Part model, mm, in its own coordinate system. A direction names the side the tool comes from. Round coordinates to 2 decimals unless told otherwise and drop trailing zeros. Order: outer loops, then holes, each group sorted by start corner. A loop starts at its lowest first (then second) coordinate and runs counter-clockwise, first axis right, second up. Notation, with made-up numbers: (74.25, -17) -> (117.25, -17) arc R12 cw to (117.25, -10) -> close; hole circle Ø10 at (38.25, 72). An arc over 180 degrees is marked (long way). Answer as a JSON object with one key per item and string values. Group by question number.
```python
from build123d import *

# Parameters (mm, degrees)
BRACKET_PLATE_DEPTH        = 10
UPPER_PIVOT_BOSS_DEPTH     = 13.5
UPPER_PIVOT_BORE_PROFILE_R = 9
UPPER_PIVOT_BORE_18_DEPTH  = 27
LOWER_PIVOT_BOSS_DEPTH     = 13.5
LOWER_PIVOT_BORE_PROFILE_R = 10
LOWER_PIVOT_BORE_20_DEPTH  = 27
STOP_LUG_DEPTH             = 13.5
PLATE_FILLET_R10_R         = 10


with BuildPart() as part:
    # Bracket Plate Profile → Bracket Plate (new body)
    with BuildSketch(Plane.XY):
        with BuildLine():
            Line((-32, 0), (-32, -68))
            Line((-32, -68), (0, -106.5))
            Line((0, -106.5), (116.5, -106.5))
            Line((116.5, -106.5), (116.5, -58.5))
            Line((116.5, -58.5), (88.5, -58.5))
            Line((88.5, -58.5), (88.5, -68.5))
            ThreePointArc((88.5, -68.5), (83.524922359, -76.549844719), (74.1, -75.7))
            Line((74.1, -75.7), (23.7, -37.9))
            ThreePointArc((23.7, -37.9), (21.602252409, -35.552292952), (20.572822936, -32.576969725))
            Line((20.572822936, -32.576969725), (15.854354129, 2.15393945))
            ThreePointArc((15.854354129, 2.15393945), (10.524660774, 12.051203907), (0, 16))
            Line((0, 16), (0, 32))
            ThreePointArc((0, 32), (-22.627416998, 22.627416998), (-32, 0))
        make_face()
    extrude(amount=BRACKET_PLATE_DEPTH)

    # Upper Pivot Boss Profile → Upper Pivot Boss (add, symmetric)
    with BuildSketch(Plane.XY.offset(5)):
        with BuildLine():
            Line((0, 16), (0, 32))
            ThreePointArc((0, 32), (-8.282209443, 30.909626441), (-16, 27.712812921))
            Line((-16, 27.712812921), (-16, 0))
            ThreePointArc((-16, 0), (11.313708499, -11.313708499), (0, 16))
        make_face()
    extrude(amount=UPPER_PIVOT_BOSS_DEPTH, both=True)

    # Upper Pivot Bore Profile → Upper Pivot Bore Ø18 (cut)
    with BuildSketch(Plane.XY.offset(18.5)):
        Circle(UPPER_PIVOT_BORE_PROFILE_R)
    extrude(amount=-UPPER_PIVOT_BORE_18_DEPTH, mode=Mode.SUBTRACT)

    # Lower Pivot Boss Profile → Lower Pivot Boss (add, symmetric)
    with BuildSketch(Plane.XY.offset(5)):
        with BuildLine():
            Line((-48.20516756, -74.470038503), (-28.953878866, -88.470038503))
            ThreePointArc((-28.953878866, -88.470038503), (-29.600430512, -76.053648048), (-17.320508076, -78))
            ThreePointArc((-17.320508076, -78), (20, -68), (-17.320508076, -58))
            ThreePointArc((-17.320508076, -58), (-29.600430512, -59.946351952), (-28.953878866, -47.529961497))
            Line((-28.953878866, -47.529961497), (-48.20516756, -61.529961497))
            ThreePointArc((-48.20516756, -61.529961497), (-51.5, -68), (-48.20516756, -74.470038503))
        make_face()
    extrude(amount=LOWER_PIVOT_BOSS_DEPTH, both=True)

    # Lower Pivot Bore Profile → Lower Pivot Bore Ø20 (cut)
    with BuildSketch(Plane.XY.offset(18.5)):
        with Locations((0, -68)):
            Circle(LOWER_PIVOT_BORE_PROFILE_R)
    extrude(amount=-LOWER_PIVOT_BORE_20_DEPTH, mode=Mode.SUBTRACT)

    # Stop Lug Profile → Stop Lug (add, symmetric)
    with BuildSketch(Plane.XY.offset(5)):
        with BuildLine():
            Line((116.5, -58.5), (116.5, -50.5))
            Line((116.5, -50.5), (128.5, -50.5))
            Line((128.5, -50.5), (111.797390872, -15.731800611))
            ThreePointArc((111.797390872, -15.731800611), (98.941207721, -11.564507441), (91, -22.5))
            Line((91, -22.5), (88.5, -58.5))
            Line((88.5, -58.5), (116.5, -58.5))
        make_face()
    extrude(amount=STOP_LUG_DEPTH, both=True)

    # Plate Fillet R10
    plate_fillet_r10_edges = [part.edges().sort_by_distance(p)[0] for p in [
        (116.5, -106.5, 5),
    ]]
    fillet(plate_fillet_r10_edges, radius=PLATE_FILLET_R10_R)


solid = part.part
```
Q1. Band-saw the part on A-A (z = -3.5). List the corners of the cut face in (x, y).
Q2. Band-saw the part on D-D (x = 71.5). List the corners of the cut face in (y, z), plus the area to 4 significant figures.
Q3. Band-saw the part on B-B (y = -82). List the corners of the cut face in (x, z).
Q4. Two-plate mould, pull along X, no slides. Class faces 5 (the flat face through (89.768, -40.248, 5.189)), 6 (the flat face through (102, -58.5, -4)), 7 (the cylindrical face through (113.65, -103.49, 5.07)): +X half, -X half, draft (parallel to the pull), parting line (faces both ways), or undercut.
Q5. Wall check: line 1 (Y direction, x = -3.5, z = 12.25); line 2 (X direction, y = -75, z = 16) (3 decimals); line 3 (X direction, y = -54, z = 13). Give the ranges that are in metal, low to high. Write a range as [from, to].
Q6. Drop flat-ended pins along their axis: pin 1 Ø4 at (x, z) = (104.5, 14) entering from -Y; pin 2 Ø5 at (y, z) = (-61.5, 6) entering from -X; pin 3 Ø4 at (x, z) = (99, 3) entering from +Y. Give the stop position or say it passes through.
Q7. Band-saw the part on C-C (y = -54). List the corners of the cut face in (x, z).
Q8. Which spindle directions (+Z, -Z, +X, -X, +Y, -Y) get a long thin tool onto all of the face, cutting with end or side? Do faces 1 (the flat face through (-16, 14, -4)), 2 (the cylindrical face through (19.987, -68.733, 14.31)), 3 (the flat face through (116.5, -69, 5)), 4 (the cylindrical face through (-32.23, -54.57, 5.19)). Say none if no direction does.
Completed:
{
 "1": {"outline": "(-48.21, -74.47) -> (-28.95, -88.47) arc R8 cw (long way) to (-17.32, -78) arc R20 ccw (long way) to (-17.32, -58) arc R8 cw (long way) to (-28.95, -47.53) -> (-48.21, -61.53) arc R8 ccw to start; (-16, 0) arc R16 ccw (long way) to (0, 16) -> (0, 32) arc R32 ccw to (-16, 27.71) -> close; (88.5, -58.5) -> (116.5, -58.5) -> (116.5, -50.5) -> (128.5, -50.5) -> (111.8, -15.73) arc R11.5 ccw to (91, -22.5) -> close; hole circle Ø20 at (0, -68); hole circle Ø18 at (0, 0)"},
 "2": {"outline": "(-106.5, 0) -> (-73.75, 0) -> (-73.75, 10) -> (-106.5, 10) -> close", "area": "327.5 mm2"},
 "3": {"outline": "(-37.85, -8.5) -> (-32.25, -8.5) -> (-32.25, 18.5) -> (-37.85, 18.5) -> close; (-20.36, 0) -> (-14.28, 0) -> (-14.28, -8.5) -> (14.28, -8.5) -> (14.28, 0) -> (116.5, 0) -> (116.5, 10) -> (14.28, 10) -> (14.28, 18.5) -> (-14.28, 18.5) -> (-14.28, 10) -> (-20.36, 10) -> close"},
 "4": {"face 5": "undercut", "face 6": "draft", "face 7": "+X half"},
 "5": {"line 1": "[-87.69, -77.37], [-58.63, -48.31], [-15.61, -8.29], [8.29, 31.81]", "line 2": "[-47.476, -28.122], [-20.376, -7.141], [7.141, 18.735]", "line 3": "[-37.85, -32.25], [-14.28, 14.28], [88.81, 116.5]"},
 "6": {"pin 1": "y = -58.5", "pin 2": "x = -50.43", "pin 3": "y = -11.1"},
 "7": {"outline": "(-37.85, -8.5) -> (-32.25, -8.5) -> (-32.25, 18.5) -> (-37.85, 18.5) -> close; (-32, 0) -> (-14.28, 0) -> (-14.28, -8.5) -> (14.28, -8.5) -> (14.28, 0) -> (45.17, 0) -> (45.17, 10) -> (14.28, 10) -> (14.28, 18.5) -> (-14.28, 18.5) -> (-14.28, 10) -> (-32, 10) -> close; (88.81, -8.5) -> (116.5, -8.5) -> (116.5, 18.5) -> (88.81, 18.5) -> close"},
 "8": {"face 1": "-Z, -X, +Y", "face 2": "+Z", "face 3": "+Z, -Z, +X, -Y", "face 4": "none"}
}
